Geometry: see drawing. Coordinates: mm, zero at the bounding-box minimum. Coordinates: 2 decimals unless noted, no trailing zeros. Order: outer loops, then holes, each group sorted by start corner. A loop starts at its lowest first (then second) coordinate and runs counter-clockwise, first axis right, second up. Notation, with made-up numbers: M 16,26 L 57,26 A5 cw 57,35 Z; hole C 13.5,-25.5 d5. An arc over 180 degrees is marked long. One line per item, written item: value.
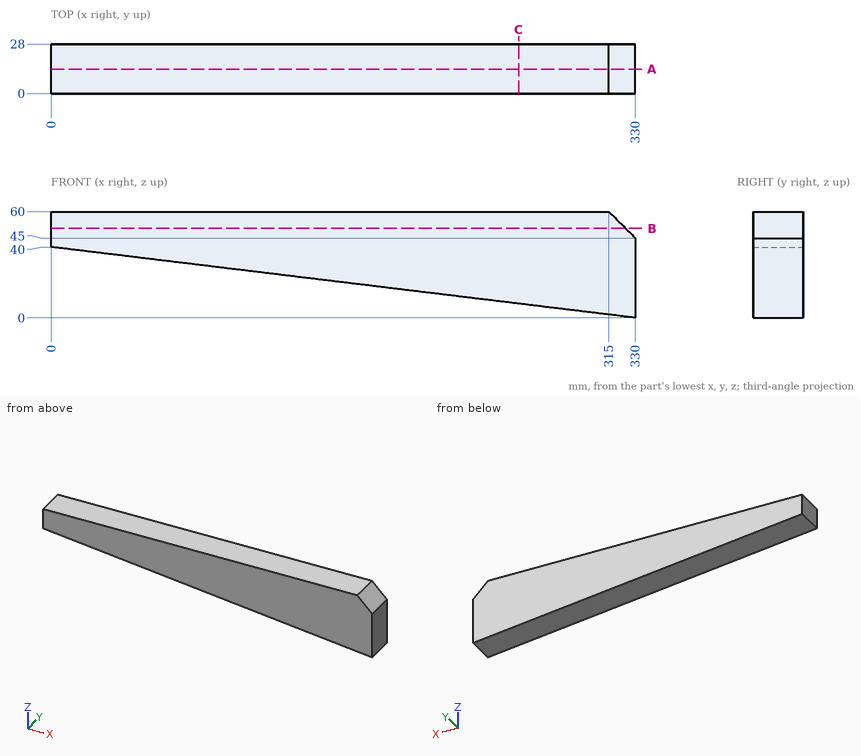
(1) Cut plane C-C on x = 264. Output: boundary loops of the cut face in (y, z).
Data:
outline: M 0,8 L 28,8 L 28,60 L 0,60 Z
(2) First-contact query: pin 1 (12 mm diameter, centred on x = 184, z = 28.5, fed in from -Y); pin 2 (1.5 mm diameter, centred on x = 132, y = 22.5, fed in from -Z). Flat tips, straight axial feed; report the tip coordinate or a pass-through.
Data:
pin 1: stops at y = 0
pin 2: stops at z = 23.91
(3) Cut plane A-A on y = 13.75. Output: boundary loops of the cut face in (x, z), plus the area to 3 significant figures.
Data:
outline: M 0,40 L 330,0 L 330,45 L 315,60 L 0,60 Z
area: 13,100 mm2
(4) Cut plane B-B on z = 50.5. Output: boundary loops of the cut face in (x, y).
Data:
outline: M 0,0 L 324.5,0 L 324.5,28 L 0,28 Z
(5) Ray query, line 1 (Z direction, x = 238, y = 9); line 2 (X direction, y = 12.75, z = 52.5); line 3 (X direction, y = 9, z = 52). Return the intervals inside material, ascending. Write a range as from..to.
Data:
line 1: z = 11.15..60
line 2: x = 0..322.5
line 3: x = 0..323
